Could you check a few things on this model? Use its own coordinates, in mm. Face numbers are marked on the shaded views. A direction names the side the tool comes from. Round coordinates to 2 decimals unless told otherwise and drop trailing zeros. Order: outer loops, then holes, each group sorted by start corner. A loop starts at its lowest first (then second) coordinate and runs counter-clockwise, first axis right, second up. Notation, with made-up numbers: (-10, 48.25) - (47, 48.25) arc R10 ccw to (47, 67.25) - close; hole circle Ø4 at (24.5, -22.75). An arc over 180 degrees is marked (long way). Return JSON: item names as keys, results as strings. Group by question number.
from build123d import *

# Parameters (mm, degrees)
SKETCH1_W                 = 600
SKETCH1_H                 = 1200
BOSS_EXTRUDE1_DEPTH       = 30
SKETCH3_W                 = 600
SKETCH3_H                 = 1200
SKETCH3_W_2               = 540
SKETCH3_H_2               = 1140
BOSS_EXTRUDE2_DEPTH       = 250
SKETCH4_R                 = 30
CUT_EXTRUDE2_DEPTH        = 660
LPATTERN1_COUNT           = 4
LPATTERN1_PITCH           = 220
SKETCH5_R                 = 5
CUT_EXTRUDE3_DEPTH        = 20
LPATTERN2_COUNT           = 4
LPATTERN2_PITCH           = 190
LPATTERN3_COUNT           = 4
LPATTERN3_PITCH           = 390
LPATTERN4_COPY_1_SKETCH_R = 5
LPATTERN4_COPY_1_DEPTH    = 20
LPATTERN4_COPY_2_SKETCH_R = 5
LPATTERN4_COPY_2_DEPTH    = 20
LPATTERN4_COPY_3_SKETCH_R = 5
LPATTERN4_COPY_3_DEPTH    = 20
LPATTERN4_COPY_4_SKETCH_R = 5
LPATTERN4_COPY_4_DEPTH    = 20
LPATTERN5_COPY_1_SKETCH_R = 5
LPATTERN5_COPY_1_DEPTH    = 20
LPATTERN5_COPY_2_SKETCH_R = 5
LPATTERN5_COPY_2_DEPTH    = 20
LPATTERN5_COPY_3_SKETCH_R = 5
LPATTERN5_COPY_3_DEPTH    = 20
LPATTERN5_COPY_4_SKETCH_R = 5
LPATTERN5_COPY_4_DEPTH    = 20
SKETCH6_W                 = 600
SKETCH6_H                 = 30
BOSS_EXTRUDE3_DEPTH       = 480
SKETCH8_W                 = 600
SKETCH8_H                 = 30
BOSS_EXTRUDE4_DEPTH       = 480
SKETCH9_R                 = 32
CUT_EXTRUDE4_DEPTH        = 480


with BuildPart() as part:
    # Sketch1 → Boss-Extrude1 (new body)
    with BuildSketch(Plane.XY):
        Rectangle(SKETCH1_W, SKETCH1_H)
    extrude(amount=BOSS_EXTRUDE1_DEPTH)

    # Sketch3 → Boss-Extrude2 (add)
    with BuildSketch(Plane(origin=(0, 0, 0), x_dir=(-1, 0, 0), z_dir=(0, 0, -1))):
        Rectangle(SKETCH3_W, SKETCH3_H)
        Rectangle(SKETCH3_W_2, SKETCH3_H_2, mode=Mode.SUBTRACT)
    extrude(amount=BOSS_EXTRUDE2_DEPTH)

    # Sketch4 → Cut-Extrude2 (cut)
    with BuildSketch(Plane.ZY.offset(300)):
        with Locations((-125, 340)):
            Circle(SKETCH4_R)
    cut_extrude2 = extrude(amount=-CUT_EXTRUDE2_DEPTH, mode=Mode.SUBTRACT)

    # LPattern1: Cut-Extrude2 ×4
    with Locations(*[(0, -i * LPATTERN1_PITCH, 0) for i in range(1, LPATTERN1_COUNT)]):
        add(cut_extrude2, mode=Mode.SUBTRACT)

    # Sketch5 → Cut-Extrude3 (cut)
    with BuildSketch(Plane(origin=(0, 0, -250), x_dir=(-1, 0, 0), z_dir=(0, 0, -1))):
        with Locations((-285, 585)):
            Circle(SKETCH5_R)
    cut_extrude3 = extrude(amount=-CUT_EXTRUDE3_DEPTH, mode=Mode.SUBTRACT)

    # LPattern2: Cut-Extrude3 ×4
    with Locations(*[(-i * LPATTERN2_PITCH, 0, 0) for i in range(1, LPATTERN2_COUNT)]):
        add(cut_extrude3, mode=Mode.SUBTRACT)

    # LPattern3: Cut-Extrude3 ×4
    with Locations(*[(0, -i * LPATTERN3_PITCH, 0) for i in range(1, LPATTERN3_COUNT)]):
        add(cut_extrude3, mode=Mode.SUBTRACT)

    # LPattern4 copy 1 sketch → LPattern4 copy 1 (cut)
    with BuildSketch(Plane(origin=(-570, -390, -250), x_dir=(-1, 0, 0), z_dir=(0, 0, -1))):
        with Locations((-285, 585)):
            Circle(LPATTERN4_COPY_1_SKETCH_R)
    extrude(amount=-LPATTERN4_COPY_1_DEPTH, mode=Mode.SUBTRACT)

    # LPattern4 copy 2 sketch → LPattern4 copy 2 (cut)
    with BuildSketch(Plane(origin=(-570, -780, -250), x_dir=(-1, 0, 0), z_dir=(0, 0, -1))):
        with Locations((-285, 585)):
            Circle(LPATTERN4_COPY_2_SKETCH_R)
    extrude(amount=-LPATTERN4_COPY_2_DEPTH, mode=Mode.SUBTRACT)

    # LPattern4 copy 3 sketch → LPattern4 copy 3 (cut)
    with BuildSketch(Plane(origin=(-570, -1170, -250), x_dir=(-1, 0, 0), z_dir=(0, 0, -1))):
        with Locations((-285, 585)):
            Circle(LPATTERN4_COPY_3_SKETCH_R)
    extrude(amount=-LPATTERN4_COPY_3_DEPTH, mode=Mode.SUBTRACT)

    # LPattern4 copy 4 sketch → LPattern4 copy 4 (cut)
    with BuildSketch(Plane(origin=(-570, 0, -250), x_dir=(-1, 0, 0), z_dir=(0, 0, -1))):
        with Locations((-285, 585)):
            Circle(LPATTERN4_COPY_4_SKETCH_R)
    extrude(amount=-LPATTERN4_COPY_4_DEPTH, mode=Mode.SUBTRACT)

    # LPattern5 copy 1 sketch → LPattern5 copy 1 (cut)
    with BuildSketch(Plane(origin=(-190, -1170, -250), x_dir=(-1, 0, 0), z_dir=(0, 0, -1))):
        with Locations((-285, 585)):
            Circle(LPATTERN5_COPY_1_SKETCH_R)
    extrude(amount=-LPATTERN5_COPY_1_DEPTH, mode=Mode.SUBTRACT)

    # LPattern5 copy 2 sketch → LPattern5 copy 2 (cut)
    with BuildSketch(Plane(origin=(-380, -1170, -250), x_dir=(-1, 0, 0), z_dir=(0, 0, -1))):
        with Locations((-285, 585)):
            Circle(LPATTERN5_COPY_2_SKETCH_R)
    extrude(amount=-LPATTERN5_COPY_2_DEPTH, mode=Mode.SUBTRACT)

    # LPattern5 copy 3 sketch → LPattern5 copy 3 (cut)
    with BuildSketch(Plane(origin=(-570, -1170, -250), x_dir=(-1, 0, 0), z_dir=(0, 0, -1))):
        with Locations((-285, 585)):
            Circle(LPATTERN5_COPY_3_SKETCH_R)
    extrude(amount=-LPATTERN5_COPY_3_DEPTH, mode=Mode.SUBTRACT)

    # LPattern5 copy 4 sketch → LPattern5 copy 4 (cut)
    with BuildSketch(Plane(origin=(0, -1170, -250), x_dir=(-1, 0, 0), z_dir=(0, 0, -1))):
        with Locations((-285, 585)):
            Circle(LPATTERN5_COPY_4_SKETCH_R)
    extrude(amount=-LPATTERN5_COPY_4_DEPTH, mode=Mode.SUBTRACT)

    # Sketch6 → Boss-Extrude3 (add)
    with BuildSketch(Plane.XZ.offset(600)):
        with Locations((0, 15)):
            Rectangle(SKETCH6_W, SKETCH6_H)
    extrude(amount=BOSS_EXTRUDE3_DEPTH)

    # Sketch8 → Boss-Extrude4 (add)
    with BuildSketch(Plane(origin=(0, 600, 0), x_dir=(1, 0, 0), z_dir=(0, 1, 0))):
        with Locations((0, -15)):
            Rectangle(SKETCH8_W, SKETCH8_H)
    extrude(amount=BOSS_EXTRUDE4_DEPTH)

    # Sketch9 → Cut-Extrude4 (cut)
    with BuildSketch(Plane.XY.offset(30)):
        with Locations((0, 880)):
            Circle(SKETCH9_R)
        with Locations((0, -880)):
            Circle(SKETCH9_R)
    extrude(amount=-CUT_EXTRUDE4_DEPTH, mode=Mode.SUBTRACT)


solid = part.part
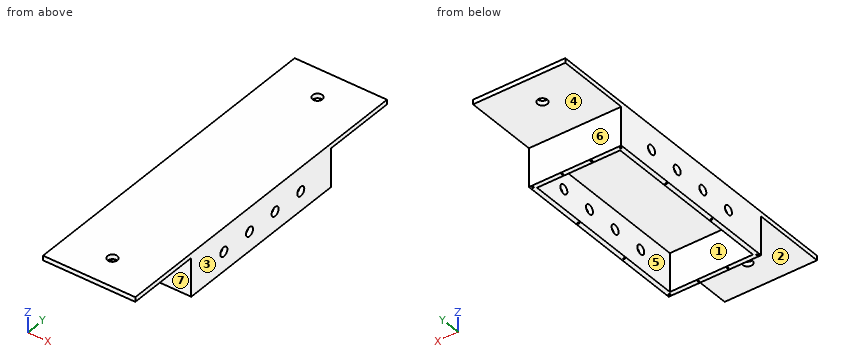
1) For the marked faces 1, 2, 3 and 4, which set-ups out of +Z, -Z, +X, -X, +Y, -Y let a thin tool reach every point of the face, with its end or its side?
2) I want a section at D-D, the plane z = -200. List the corners of the cut face in (x, y) for me, plus the area to 3 significant figures.
3) I want a section at A-A, the plane x = 0. List the corners of the cut face in (y, z) for me.
4) We'd pull the mould along Y, two halves only. Please class the marked faces 5, 6 and 7: +Y half, -Y half, draft (parallel to the pull), parting line (faces both ways), or undercut.
5) Will these pins go through, and if not, where does the flat tip stop? pin 1 (8 mm diameter, centred on x = -285, y = -195, fed in from -Z); pin 2 (8 mm diameter, centred on x = 97, y = 11.5, fed in from -Z); pin 3 (1.5 mm diameter, centred on x = 171.5, z = -31.5, fed in from -Y).
6) If I drill on line 1 along Y through (x, z) = (285, -240); line 2 along Y through (x, z) = (-95, -243); line 3 along X through (y, z) = (-173, -64.5), over which ranges is the centre line in solid material (lowest first)? Write a range as from..to.
7) I want a section at B-B, the plane y = -880. List the corners of the cut face in (x, z) for me.
8) I want a section at C-C, the plane y = -100. List the corners of the cut face in (x, z) for me, plus the area to 3 significant figures.
Outcome:
{
 "1": {"face 1": "-Z", "face 2": "-Z, +X, -X, -Y", "face 3": "+Z, -Z, +X, +Y, -Y", "face 4": "-Z, +X, -X, +Y"},
 "2": {"outline": "(-300, -600) - (300, -600) - (300, 600) - (-300, 600) - close; hole (-270, -570) - (270, -570) - (270, 570) - (-270, 570) - close", "area": "104,000 mm^2"},
 "3": {"outline": "(-1080, 0) - (-912, 0) - (-912, 30) - (-1080, 30) - close; (-848, 0) - (-600, 0) - (-600, -250) - (-570, -250) - (-570, 0) - (570, 0) - (570, -250) - (600, -250) - (600, 0) - (848, 0) - (848, 30) - (-848, 30) - close; (912, 0) - (1080, 0) - (1080, 30) - (912, 30) - close"},
 "4": {"face 5": "undercut", "face 6": "+Y half", "face 7": "-Y half"},
 "5": {"pin 1": "z = -230", "pin 2": "z = 0", "pin 3": "y = -600"},
 "6": {"line 1": "-600..-590, -580..-200, -190..190, 200..580, 590..600", "line 2": "-600..-590, -580..-570, 570..580, 590..600", "line 3": "-300..-270, 270..300"},
 "7": {"outline": "(-300, 0) - (-32, 0) - (-32, 30) - (-300, 30) - close; (32, 0) - (300, 0) - (300, 30) - (32, 30) - close"},
 "8": {"outline": "(-300, -250) - (-270, -250) - (-270, -155) - (-300, -155) - close; (-300, -95) - (-270, -95) - (-270, 0) - (270, 0) - (270, -95) - (300, -95) - (300, 30) - (-300, 30) - close; (270, -250) - (300, -250) - (300, -155) - (270, -155) - close", "area": "29,400 mm^2"}
}
